Design review of the part built by this model. Coordinates are the model's own, in mm. Face numbers are marked on the shaded views. Coordinates: 2 decimals unless noted, no trailing zeros. Write each loop counter-clockwise with the first axis right and the second up, starting at its lowest first coordinate (ties: lowest second). Pieces come first, ordered by that corner, then holes.
Q1. Take a section at C-C, the plane y = 10. Write out the cut boundary in (x, z), plus the area to 3 significant figures.
Q2. The part is to be moulded in two halves that separate along X. For the marked faces 1 and 2, say which applies: released by +X, released by -X, zero draft, split by the parting line, or undercut.
Q3. For pin 1 Ø5 at (x, y) = (0, -9.5) entering from -Z; pin 2 Ø5 at (x, z) = (-2, 120.5) entering from +Y; pin 3 Ø5 at (y, z) = (-5, 136) entering from +X; pin 4 Ø1.5 at (y, z) = (-12, 86.5) entering from +X, all flat-tipped, find the tip position at first contact; note any pin that passes through.
Q4. Take a section at B-B, the plane z = 116. Write out the cut boundary in (x, y), plus the area to 3 significant figures.
Q5. Take a section at A-A, the plane x = 0. Write out the cut boundary in (y, z), plus the area to 3 significant figures.
Q6. For L1, parallel to X at y = -1, z = 76.5; L2, parallel to X at y = 10.5, z = 12.5; L3, parallel to X at y = 17.5, z = 108.5, list the stretches that pass through material, from the lowest coordinate up.
Q7. Take a section at D-D, the plane z = 63. Write out the cut boundary in (x, y).
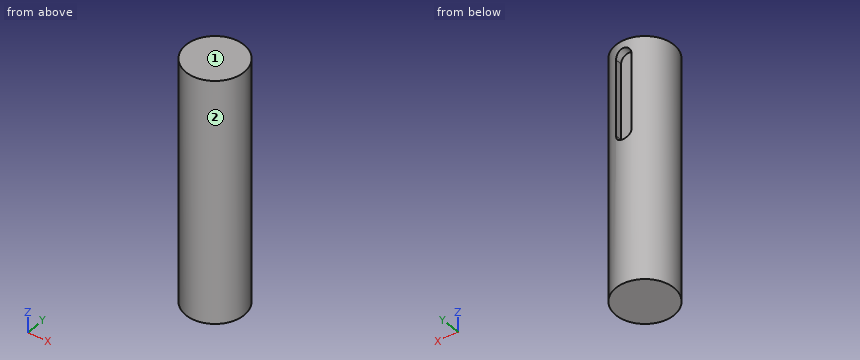
from build123d import *

# Parameters (mm, degrees)
SKETCH_1_R           = 19
BOSS_EXTRUDE_1_DEPTH = 160
CUT_EXTRUDE_1_DEPTH  = 165.468842034


with BuildPart() as part:
    # Sketch 1 → Boss-Extrude 1 (new body)
    with BuildSketch(Plane.XY):
        Circle(SKETCH_1_R)
    extrude(amount=BOSS_EXTRUDE_1_DEPTH)

    # Sketch 3 → Cut-Extrude 1 (cut, through all)
    with BuildSketch(Plane(origin=(0, 14, 0), x_dir=(1, 0, 0), z_dir=(0, 1, 0))):
        with BuildLine():
            Line((-5, -150), (-5, -100))
            ThreePointArc((-5, -100), (0, -95), (5, -100))
            Line((5, -100), (5, -150))
            ThreePointArc((5, -150), (0, -155), (-5, -150))
        make_face()
    extrude(amount=CUT_EXTRUDE_1_DEPTH, mode=Mode.SUBTRACT)


solid = part.part
Responses:
1. outline: (-16.16, 0) - (16.16, 0) - (16.16, 160) - (-16.16, 160) - close
1. area: 5,170 mm2
2. face 1: zero draft
2. face 2: split by the parting line
3. pin 1: stops at z = 0
3. pin 2: stops at y = 14
3. pin 3: stops at x = 18.83
3. pin 4: stops at x = 15.31
4. outline: (-5, 14) - (-5, 18.33) arc R19 ccw (long way) to (5, 18.33) - (5, 14) - close
4. area: 1,090 mm2
5. outline: (-19, 0) - (19, 0) - (19, 95) - (14, 95) - (14, 155) - (19, 155) - (19, 160) - (-19, 160) - close
5. area: 5,780 mm2
6. L1: x = -18.97 to 18.97
6. L2: x = -15.84 to 15.84
6. L3: x = -7.4 to -5, 5 to 7.4
7. outline: circle Ø38 at (0, 0)
